from build123d import *

# Parameters (mm, degrees)
SKETCH1_W           = 500
SKETCH1_H           = 400
BOSS_EXTRUDE1_DEPTH = 20
SKETCH2_W           = 52
SKETCH2_H           = 300
BOSS_EXTRUDE2_DEPTH = 50
SKETCH3_W           = 300
SKETCH3_H           = 400
BOSS_EXTRUDE3_DEPTH = 40
SKETCH6_R           = 75
BOSS_EXTRUDE5_DEPTH = 73
SKETCH7_R           = 15
CUT_EXTRUDE2_DEPTH  = 456.768581629


with BuildPart() as part:
    # Sketch1 → Boss-Extrude1 (new body)
    with BuildSketch(Plane(origin=(0, 0, 0), x_dir=(1, 0, 0), z_dir=(0, 1, 0))):
        Rectangle(SKETCH1_W, SKETCH1_H)
    extrude(amount=BOSS_EXTRUDE1_DEPTH)

    # Sketch2 → Boss-Extrude2 (add)
    with BuildSketch(Plane(origin=(0, 20, 0), x_dir=(1, 0, 0), z_dir=(0, 1, 0))):
        with Locations((-96, -50)):
            Rectangle(SKETCH2_W, SKETCH2_H)
        with Locations((96, -50)):
            Rectangle(SKETCH2_W, SKETCH2_H)
    extrude(amount=BOSS_EXTRUDE2_DEPTH)

    # Sketch3 → Boss-Extrude3 (add)
    with BuildSketch(Plane.XZ):
        Rectangle(SKETCH3_W, SKETCH3_H)
    extrude(amount=BOSS_EXTRUDE3_DEPTH)

    # Sketch6 → Boss-Extrude5 (add)
    with BuildSketch(Plane.XY.offset(160)):
        with Locations((0, 50)):
            Circle(SKETCH6_R)
    extrude(amount=-BOSS_EXTRUDE5_DEPTH)

    # Sketch7 → Cut-Extrude2 (cut, through all)
    with BuildSketch(Plane.XY.offset(160)):
        with Locations((0, 50)):
            Circle(SKETCH7_R)
    extrude(amount=-CUT_EXTRUDE2_DEPTH, mode=Mode.SUBTRACT)


solid = part.part
Design review of the part built by this model. Coordinates are the model's own, in mm. A direction names the side the tool comes from. Round coordinates to 2 decimals unless told otherwise and drop trailing zeros. Loops run counter-clockwise (first coordinate to the right, second up) from the corner with the lowest first, then second, coordinate; pieces in that order, holes last. Notation, with made-up numbers: (71, 88) - (90, 88) arc R26 ccw to (90, 119) - close; hole circle Ø10 at (-33.75, -6.75). An arc over 180 degrees is marked (long way). One line per item, written item: value. Start each with the question number.
1) Consider section C-C on z = -71. Give the boundary of the cut face in (x, y), then the cut area to 3 significant figures.
2) To check wall thickness, follow L1, parallel to X at y = 58, z = 0; L2, parallel to Y at x = 0, z = 138; L3, parallel to Y at x = -36.5, z = -92. State the ranges of each line that lie inside material, in increasing order. Write a range as from..to.
3) Draft analysis for pull direction X (two halves, no side actions). For faces 6 (the flat face through (70, 45, 19)), 7 (the flat face through (150, -20, -3)), 8 (the flat face through (-150, -20, -3)), state which applies: +X half, -X half, draft (parallel to the pull), parting line (faces both ways), or undercut.
4) For faces 1 (the flat face through (-122, 45, 52)), 2 (the flat face through (-96, 45, -100)), 3 (the cylindrical face through (1.366, 124.988, 124.011)), 4 (the flat face through (-201, 0, -3)), 5 (the flat face through (-3, -4, -200)), list the 3-axis set-ups (+Z, -Z, +X, -X, +Y, -Y) from which the entire face can be reached by the end or side of a thin tool; tool diameter is ignored.
5) Consider section B-B on x = 0. Give the boundary of the cut face in (y, z), then the cut area to 3 significant figures.
6) Insertion check: pin 1 Ø8 at (x, z) = (-131, -97) entering from +Y; pin 2 Ø25 at (x, y) = (-100.5, 49.5) entering from -Z; pin 3 Ø15 at (y, z) = (47, 19.5) entering from -X. Each pin has a flat end and moves straight along its axis. Give the tip position at first contact, or say it passes through.
7) Consider section D-D on x = -82. Give the boundary of the cut face in (y, z), then the cut area to 3 significant figures.
8) Consider section A-A on y = 50. Give the boundary of the cut face in (x, z).
Reported:
1. outline: (-250, 0) - (-150, 0) - (-150, -40) - (150, -40) - (150, 0) - (250, 0) - (250, 20) - (122, 20) - (122, 70) - (70, 70) - (70, 20) - (-70, 20) - (-70, 70) - (-122, 70) - (-122, 20) - (-250, 20) - close
1. area: 27,200 mm^2
2. L1: x = -122..-70, 70..122
2. L2: y = -40..35, 65..125
2. L3: y = -40..20
3. face 6: undercut
3. face 7: +X half
3. face 8: -X half
4. face 1: +Z, -Z, -X, +Y
4. face 2: -Z, +X, -X, +Y
4. face 3: +Z, -Z, +Y
4. face 4: +Z, -Z, -X, -Y
4. face 5: -Z, +X, -X, +Y, -Y
5. outline: (-40, -200) - (20, -200) - (20, 87) - (35, 87) - (35, 160) - (20, 160) - (20, 200) - (-40, 200) - close; (65, 87) - (125, 87) - (125, 160) - (65, 160) - close
5. area: 29,500 mm^2
6. pin 1: stops at y = 20
6. pin 2: stops at z = -100
6. pin 3: stops at x = -122
7. outline: (-40, -200) - (20, -200) - (20, -100) - (70, -100) - (70, 200) - (-40, 200) - close
7. area: 39,000 mm^2
8. outline: (-122, -100) - (-70, -100) - (-70, 87) - (-15, 87) - (-15, 160) - (-70, 160) - (-70, 200) - (-122, 200) - close; (15, 87) - (70, 87) - (70, -100) - (122, -100) - (122, 200) - (70, 200) - (70, 160) - (15, 160) - close
